Job drawing, mm, ordinate dimensions from the low corner. One solid piece. Round coordinates to 2 decimals unless told otherwise and drop trailing zeros. Order: outer loops, then holes, each group sorted by start corner. A loop starts at its lowest first (then second) coordinate and runs counter-clockwise, first axis right, second up. Notation, with made-up numbers: (-37.75, 47) -> (-14.75, 47) arc R10 cw to (-14.75, 53) -> close; hole circle Ø6 at (75, 39.5). An arc over 180 degrees is marked (long way). Use CSV: the item, a comma, the result in double quotes.
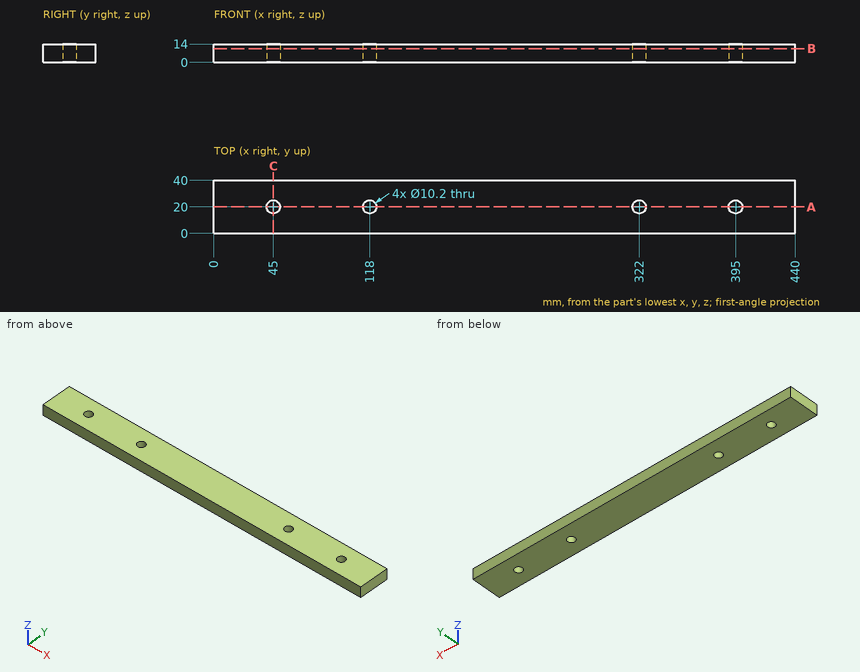
(1) Cut at B-B, the plane z = 10.5. Give the cut face in (x, y).
Reply:
outline,"(0, 0) -> (440, 0) -> (440, 40) -> (0, 40) -> close; hole circle Ø10.2 at (45, 20); hole circle Ø10.2 at (118, 20); hole circle Ø10.2 at (322, 20); hole circle Ø10.2 at (395, 20)"
(2) Probe probe 1 along Y at (x, z) = (118, 9.5); probe 2 along X at (y, z) = (17.5, 2.75); probe 3 along X at (y, z) = (21, 3.5). List the from-to ranges inside material, lowest first. Write a range as [from, to].
Reply:
probe 1,"[0, 14.9], [25.1, 40]"
probe 2,"[0, 40.55], [49.45, 113.55], [122.45, 317.55], [326.45, 390.55], [399.45, 440]"
probe 3,"[0, 40], [50, 113], [123, 317], [327, 390], [400, 440]"
(3) Cut at C-C, the plane x = 45. Give the cut face in (y, z), then the cut area to 3 significant figures.
Reply:
outline,"(0, 0) -> (14.9, 0) -> (14.9, 14) -> (0, 14) -> close; (25.1, 0) -> (40, 0) -> (40, 14) -> (25.1, 14) -> close"
area,"417 mm2"
(4) Cut at A-A, the plane y = 20. Give the cut face in (x, z).
Reply:
outline,"(0, 0) -> (39.9, 0) -> (39.9, 14) -> (0, 14) -> close; (50.1, 0) -> (112.9, 0) -> (112.9, 14) -> (50.1, 14) -> close; (123.1, 0) -> (316.9, 0) -> (316.9, 14) -> (123.1, 14) -> close; (327.1, 0) -> (389.9, 0) -> (389.9, 14) -> (327.1, 14) -> close; (400.1, 0) -> (440, 0) -> (440, 14) -> (400.1, 14) -> close"
(5) Drop a flat-ended pin along its axis: P1, Ø6, axis at y = 35.5, z = 2.5, coming from the -X side. Give the stop position or say it passes through.
Reply:
P1,"x = 0"
